Source: CAD feature listing. Evaluate the final solid. Frame: model axes, mm. Face numbers are marked on the shaded views. A direction names the side the tool comes from. Round coordinates to 2 decimals unless told otherwise and drop trailing zeros. Order: outer loops, then holes, each group sorted by start corner. A loop starts at its lowest first (then second) coordinate and runs counter-clockwise, first axis right, second up. Notation, with made-up numbers: (-21, 38.5) - (-8, 38.5) arc R26 ccw to (-8, 76.5) - close; hole circle Ø2 at (64.25, 61). An arc over 180 degrees is marked (long way). Use one line per item in the form item = value. Start each with the question number.
Q1. Ray query, line 1 (Y direction, x = 21, z = -3); line 2 (X direction, y = -5.75, z = 4.5); line 3 (Y direction, x = 48, z = 0.25). Return the intervals inside material, ascending. Write a range as [from, to].
Q2. Cut plane A-A, the plane x = 19. Return the cut outline in (y, z).
Q3. Pin query (flat end, axial travel): pin 1 Ø3 at (x, y) = (12.5, 4.5) entering from +Z; pin 2 Ø2 at (x, y) = (26.5, 2.5) entering from +Z; pin 3 Ø0.7 at (y, z) = (-8.5, 0.5) entering from +X; pin 4 Ø3 at (y, z) = (-2, 5.5) entering from +X. Return the tip coordinate at first contact, or that it passes through.
Q4. Set-up query: the marked faces 1 and 2. Return all of +Z, -Z, +X, -X, +Y, -Y with unobstructed straight access to the full face (end or side cutting, diameter ignored); none if empty.
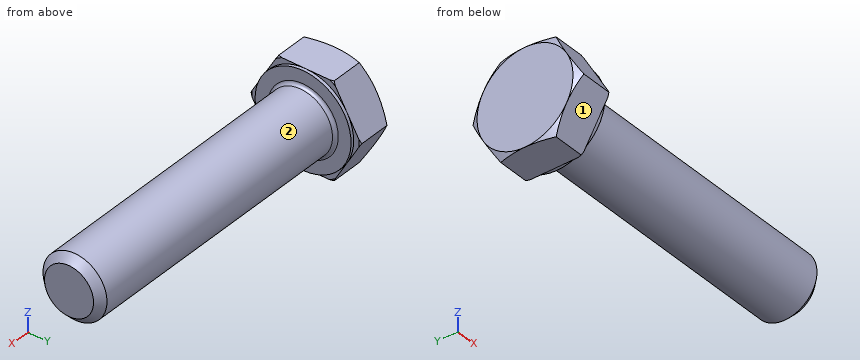
from build123d import *

# Parameters (mm, degrees)
BASE_EXTRUDE_DEPTH = 7.5
SKETCH4_W          = 0.6
SKETCH4_H          = 11.392304845
CHAMFER_2_SIZE     = 1.4
FILLET_2_R         = 0.6


with BuildPart() as part:
    # Sketch1 → Base-Extrude (new body)
    with BuildSketch(Plane(origin=(0, 0, 0), x_dir=(0, 0, -1), z_dir=(1, 0, 0))):
        Polygon((9, 5.196152423), (9, -5.196152423), (0, -10.392304845), (-9, -5.196152423), (-9, 5.196152423), (0, 10.392304845), align=None)
    extrude(amount=BASE_EXTRUDE_DEPTH)

    # Sketch2 → Boss-Revolve1 (revolve)
    with BuildSketch(Plane.XY, mode=Mode.PRIVATE) as boss_revolve1_sk:
        Polygon((0, 0), (62.5, 0), (62.5, 4.4845), (62.5, 6), (7.791693541, 6), (0, 6), align=None)
    revolve(boss_revolve1_sk.sketch.rotate(Axis((0, 0, 0), (1, 0, 0)), 90), axis=Axis((0, 0, 0), (1, 0, 0)))

    # Sketch3 → Cut-Revolve1 (revolve, cut)
    with BuildSketch(Plane.XY):
        Polygon((0, 9), (3.690598923, 15.392304845), (3.690598923, 20.392304845), (-10, 20.392304845), (-10, 9), align=None)
    revolve(axis=Axis((0, 0, 0), (1, 0, 0)), mode=Mode.SUBTRACT)

    # Sketch5 → Cut-Revolve2 (revolve, cut)
    with BuildSketch(Plane.XY):
        Polygon((7.5, 9), (3.809401077, 15.392304845), (3.809401077, 20.392304845), (13.809401077, 20.392304845), (13.809401077, 9), align=None)
    revolve(axis=Axis((0, 0, 0), (1, 0, 0)), mode=Mode.SUBTRACT)

    # Sketch4 → Cut-Revolve3 (revolve, cut)
    with BuildSketch(Plane.XY, mode=Mode.PRIVATE) as cut_revolve3_sk:
        with Locations((7.2, 14.696152423)):
            Rectangle(SKETCH4_W, SKETCH4_H)
    revolve(cut_revolve3_sk.sketch.rotate(Axis((0, 0, 0), (1, 0, 0)), 270), axis=Axis((0, 0, 0), (1, 0, 0)), mode=Mode.SUBTRACT)

    # Chamfer 2
    chamfer_2_edges = [part.edges().sort_by_distance(p)[0] for p in [
        (62.5, 0, -6),
    ]]
    chamfer(chamfer_2_edges, length=CHAMFER_2_SIZE)

    # Fillet 2
    fillet_2_edges = [part.edges().sort_by_distance(p)[0] for p in [
        (7.5, 0, -6),
    ]]
    fillet(fillet_2_edges, radius=FILLET_2_R)


solid = part.part
Completed:
q1.line_1 = [-5.2, 5.2]
q1.line_2 = [0, 7.5]
q1.line_3 = [-5.99, 5.99]
q2.outline = circle Ø12 at (0, 0)
q3.pin_1 = 5.2
q3.pin_2 = 5.81
q3.pin_3 = 7.5
q3.pin_4 = 62.5
q4.face_1 = -Z, +X, -X, -Y
q4.face_2 = +X
